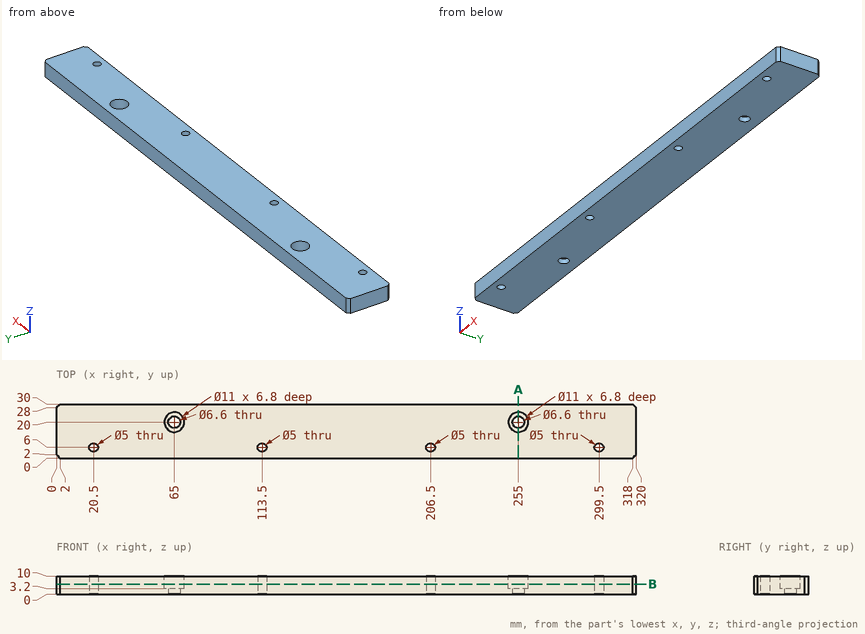
Here's the drawing with two shaded views (mm, measured from the low corner). I have some questions. Give positions to 0.01 mm unless a question says otherwise; leave off trailing zeros. Order: outer loops, then holes, each group sorted by start corner. A loop starts at its lowest first (then second) coordinate and runs counter-clockwise, first axis right, second up. Notation, with made-up numbers: M 35,-32 L 82,-32 A26 ccw 82,-1 Z; hole C 2.25,50.5 d4. An arc over 180 degrees is marked long. One line per question, with ' | ' between items.
Item 1: Suppose I cut it at B-B, the plane z = 5.75. Write out the boundary of the cut face in (x, y).
Answer block:
outline: M 0,2 L 2,0 L 318,0 L 320,2 L 320,28 L 318,30 L 2,30 L 0,28 Z; hole C 20.5,6 d5; hole C 65,20 d11; hole C 113.5,6 d5; hole C 206.5,6 d5; hole C 255,20 d11; hole C 299.5,6 d5
Item 2: Please list where these lines run through material, in increasing order: L1, parallel to Y at x = 299.5, z = 5.75; L2, parallel to Y at x = 65, z = 0.9; L3, parallel to X at y = 17, z = 7.75.
Answer block:
L1: y = 0 to 3.5, 8.5 to 30 | L2: y = 0 to 16.7, 23.3 to 30 | L3: x = 0 to 60.39, 69.61 to 250.39, 259.61 to 320
Item 3: Suppose I cut it at A-A, the plane x = 255. Write out the boundary of the cut face in (y, z), then the cut area to 3 significant figures.
Answer block:
outline: M 0,0 L 16.7,0 L 16.7,3.2 L 14.5,3.2 L 14.5,10 L 0,10 Z; M 23.3,0 L 30,0 L 30,10 L 25.5,10 L 25.5,3.2 L 23.3,3.2 Z | area: 204 mm2
Item 4: I'm going to push flat-ended pins straight in: pin 1 Ø7.5 at (x, y) = (65, 20) entering from +Z; pin 2 Ø6.5 at (x, y) = (65, 20) entering from -Z. Where does each tip first touch, or does it pass through?
Answer block:
pin 1: stops at z = 3.2 | pin 2: passes through
